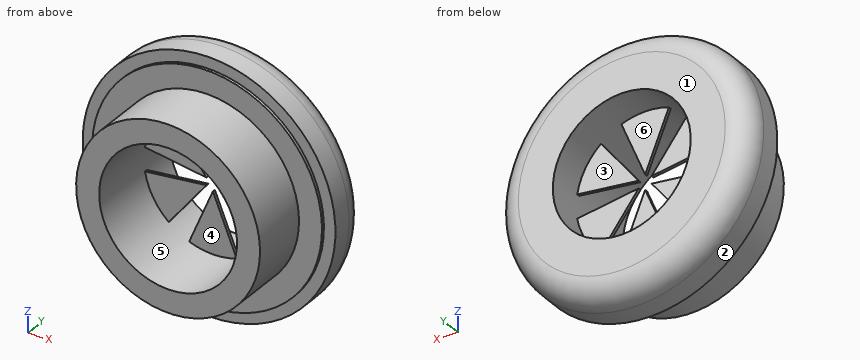
```python
from build123d import *

# Parameters (mm, degrees)
SKETCH1_R           = 8
BOSS_EXTRUDE1_DEPTH = 5
SKETCH2_R           = 11
BOSS_EXTRUDE2_DEPTH = 4
CUT_EXTRUDE1_REACH  = 19.972
SKETCH3_R           = 6
BOSS_EXTRUDE3_START = -6
BOSS_EXTRUDE3_DEPTH = 0.25
SKETCH5_R           = 11
SKETCH5_R_2         = 10
CUT_EXTRUDE2_DEPTH  = 0.25
FILLET1_R           = 2


with BuildPart() as part:
    # Sketch1 → Boss-Extrude1 (new body)
    with BuildSketch(Plane(origin=(0, 0, 0), x_dir=(1, 0, 0), z_dir=(0, 1, 0))):
        with Locations(Location((0, 0, 0), (0, 0, 270))):
            Circle(SKETCH1_R)
    extrude(amount=BOSS_EXTRUDE1_DEPTH)

    # Sketch2 → Boss-Extrude2 (add)
    with BuildSketch(Plane(origin=(0, 5, 0), x_dir=(1, 0, 0), z_dir=(0, 1, 0))):
        with Locations(Location((0, 0, 0), (0, 0, 270))):
            Circle(SKETCH2_R)
    extrude(amount=BOSS_EXTRUDE2_DEPTH)

    # Sketch3 → Cut-Extrude1 (cut, up to next)
    with BuildSketch(Plane(origin=(0, 9, 0), x_dir=(1, 0, 0), z_dir=(0, 1, 0)), mode=Mode.PRIVATE) as cut_extrude1_sk1:
        with Locations(Location((0, 0, 0), (0, 0, 270))):
            Circle(SKETCH3_R)
    cut_extrude1_tool1 = extrude(cut_extrude1_sk1.sketch, amount=-CUT_EXTRUDE1_REACH, mode=Mode.PRIVATE) & part.part
    add(cut_extrude1_tool1.solids().sort_by_distance((0, 9, 0))[0], mode=Mode.SUBTRACT)

    # Sketch4 → Boss-Extrude3 (add)
    with BuildSketch(Plane.XZ.offset(BOSS_EXTRUDE3_START)):
        with BuildLine():
            Line((0, 0.65), (-2.064316872, 5.633701789))
            ThreePointArc((-2.064316872, 5.633701789), (0, 6), (2.064316872, 5.633701789))
            Line((2.064316872, 5.633701789), (0, 0.65))
        make_face()
        with BuildLine():
            Line((0.562916512, 0.325), (3.846770431, 4.604601747))
            ThreePointArc((3.846770431, 4.604601747), (5.196152423, 3), (5.911087303, 1.029100042))
            Line((5.911087303, 1.029100042), (0.562916512, 0.325))
        make_face()
        with BuildLine():
            Line((0.562916512, -0.325), (5.911087303, -1.029100042))
            ThreePointArc((5.911087303, -1.029100042), (5.196152423, -3), (3.846770431, -4.604601747))
            Line((3.846770431, -4.604601747), (0.562916512, -0.325))
        make_face()
        with BuildLine():
            Line((0, -0.65), (2.064316872, -5.633701789))
            ThreePointArc((2.064316872, -5.633701789), (0, -6), (-2.064316872, -5.633701789))
            Line((-2.064316872, -5.633701789), (0, -0.65))
        make_face()
        with BuildLine():
            Line((-0.562916512, -0.325), (-3.846770431, -4.604601747))
            ThreePointArc((-3.846770431, -4.604601747), (-5.196152423, -3), (-5.911087303, -1.029100042))
            Line((-5.911087303, -1.029100042), (-0.562916512, -0.325))
        make_face()
        with BuildLine():
            Line((-0.562916512, 0.325), (-5.911087303, 1.029100042))
            ThreePointArc((-5.911087303, 1.029100042), (-5.196152423, 3), (-3.846770431, 4.604601747))
            Line((-3.846770431, 4.604601747), (-0.562916512, 0.325))
        make_face()
    extrude(amount=BOSS_EXTRUDE3_DEPTH)

    # Sketch5 → Cut-Extrude2 (cut)
    with BuildSketch(Plane.XZ.offset(-5)):
        with Locations(Location((0, 0, 0), (0, 0, 270))):
            Circle(SKETCH5_R)
        with Locations(Location((0, 0, 0), (0, 0, 270))):
            Circle(SKETCH5_R_2, mode=Mode.SUBTRACT)
    extrude(amount=-CUT_EXTRUDE2_DEPTH, mode=Mode.SUBTRACT)

    # Fillet1
    fillet1_edges = [part.edges().sort_by_distance(p)[0] for p in [
        (0, 9, -11),
    ]]
    fillet(fillet1_edges, radius=FILLET1_R)


solid = part.part
```
Part model, mm, in its own coordinate system. Face numbers are marked on the shaded views. A direction names the side the tool comes from. Round coordinates to 2 decimals unless told otherwise and drop trailing zeros. Write each loop counter-clockwise with the first axis right and the second up, starting at its lowest first coordinate (ties: lowest second). Pieces come first, ordered by that corner, then holes. Notation, with made-up numbers: M 36.5,-28.75 L 74.5,-28.75 A13 cw 74.5,-4.75 Z; hole C -30.75,-7 d11. An arc over 180 degrees is marked long. Answer as CSV lines item,"result". Start each with the question number.
1) Band-saw the part on A-A (z = 0). List the corners of the cut face in (x, y).
2) Band-saw the part on B-B (x = 1.5). Count the separate pieces of the cut face and the enclosed holes in it, then the cut area to 3 significant figures.
3) Drill centre lines: L1, parallel to X at y = 6.5, z = 0; L2, parallel to X at y = 3.5, z = 0.25; L3, parallel to Y at x = 7, z = -4. Where is each one in solid material? Low to high.
4) Mould opens along X. For the marked faces 1, 2 and 3 say: +X half, -X half, draft (parallel to the pull), parting line (faces both ways), or undercut.
5) Which spindle directions (+Z, -Z, +X, -X, +Y, -Y) get a long thin tool onto all of the face, cutting with end or side? Do the marked faces 4, 5 and 6. Say none if no direction does.
6) Drop flat-ended pins along their axis: pin 1 (2 mm diameter, centred on x = 4.5, z = 3, fed in from -Y); pin 2 (2 mm diameter, centred on x = 3, z = -3, fed in from +Y); pin 3 (1.5 mm diameter, centred on x = 4, y = 2, fed in from -Z); pin 4 (3.5 mm diameter, centred on x = 0, z = -3.5, fed in from -Y). Give the stop position or say it passes through.
Worked out:
1,outline,"M -11,5.25 L -10,5.25 L -10,5 L -8,5 L -8,0 L -6,0 L -6,9 L -9,9 A2 ccw -11,7 Z; M 6,0 L 8,0 L 8,5 L 10,5 L 10,5.25 L 11,5.25 L 11,7 A2 ccw 9,9 L 6,9 Z"
2,separate pieces,"4"
2,enclosed holes,"0"
2,area,"60.3 mm²"
3,L1,"-11 to -6, 6 to 11"
3,L2,"-8 to -5.99, 5.99 to 8"
3,L3,"5 to 9"
4,face 1,"draft"
4,face 2,"parting line"
4,face 3,"undercut"
5,face 4,"-Y"
5,face 5,"none"
5,face 6,"+Y"
6,pin 1,"y = 0"
6,pin 2,"y = 6"
6,pin 3,"z = -7.31"
6,pin 4,"y = 5.75"
